from build123d import *


with BuildPart() as part:
    # 草图1 → 旋转1 (revolve)
    with BuildSketch(Plane.XY, mode=Mode.PRIVATE) as revolve_1_sk:
        with BuildLine():
            Line((-2.5, 7.7), (-2.5, 6.4))
            Line((-2.5, 6.4), (-2.25, 6.4))
            Line((-2.25, 6.4), (-2.25, 5))
            Line((-2.25, 5), (-2.5, 5))
            Line((-2.5, 5), (-2.5, 2.8))
            ThreePointArc((-2.5, 2.8), (-2.412132034, 2.587867966), (-2.2, 2.5))
            Line((-2.2, 2.5), (2.2, 2.5))
            ThreePointArc((2.2, 2.5), (2.412132034, 2.587867966), (2.5, 2.8))
            Line((2.5, 2.8), (2.5, 5))
            Line((2.5, 5), (2.25, 5))
            Line((2.25, 5), (2.25, 6.4))
            Line((2.25, 6.4), (2.5, 6.4))
            Line((2.5, 6.4), (2.5, 7.7))
            ThreePointArc((2.5, 7.7), (2.412132034, 7.912132034), (2.2, 8))
            Line((2.2, 8), (-2.2, 8))
            ThreePointArc((-2.2, 8), (-2.412132034, 7.912132034), (-2.5, 7.7))
        make_face()
    revolve(revolve_1_sk.sketch.rotate(Axis((2.5, 0, 0), (-1, 0, 0)), 270), axis=Axis((2.5, 0, 0), (-1, 0, 0)))


solid = part.part
Work out the finished part from the listing and answer in its coordinate system (mm). Give positions to 0.01 mm unless a question says otherwise; leave off trailing zeros. Order: outer loops, then holes, each group sorted by start corner. A loop starts at its lowest first (then second) coordinate and runs counter-clockwise, first axis right, second up. Notation, with made-up numbers: (23.25, 88) -> (71.25, 88) arc R26 ccw to (71.25, 111) -> close; hole circle Ø10 at (83, 43). An arc over 180 degrees is marked (long way). Answer as a JSON object with one key per item and string values. Group by question number.
1. The mould has two halves that part along Z. Classify faces 1 (the flat face through (2.25, -2, 5)), 2 (the cylindrical face through (-0.03, -7.81, -1.73)), 3 (the flat face through (-2.25, -2, -5)), 4 (the flat face through (2.5, -2.2, -2.2)): released by +Z, released by -Z, zero draft, split by the parting line, or undercut.
2. Section C-C on x = -0.9 is taken. Determine the outline of the cut face in (y, z).
3. Consider line 1 along Y through (x, z) = (0.85, 0); line 2 along Y through (x, z) = (-2.35, 0); line 3 along Y through (x, z) = (2.4, 0). Determine where each line is inside the solid, lowest interval first. Write a range as [from, to].
Result sheet:
{
 "1": {"face 1": "undercut", "face 2": "split by the parting line", "face 3": "undercut", "face 4": "zero draft"},
 "2": {"outline": "circle Ø16 at (0, 0); hole circle Ø5 at (0, 0)"},
 "3": {"line 1": "y = [-8, -2.5], [2.5, 8]", "line 2": "y = [-7.96, -6.4], [-5, -2.54], [2.54, 5], [6.4, 7.96]", "line 3": "y = [-7.92, -6.4], [-5, -2.58], [2.58, 5], [6.4, 7.92]"}
}
